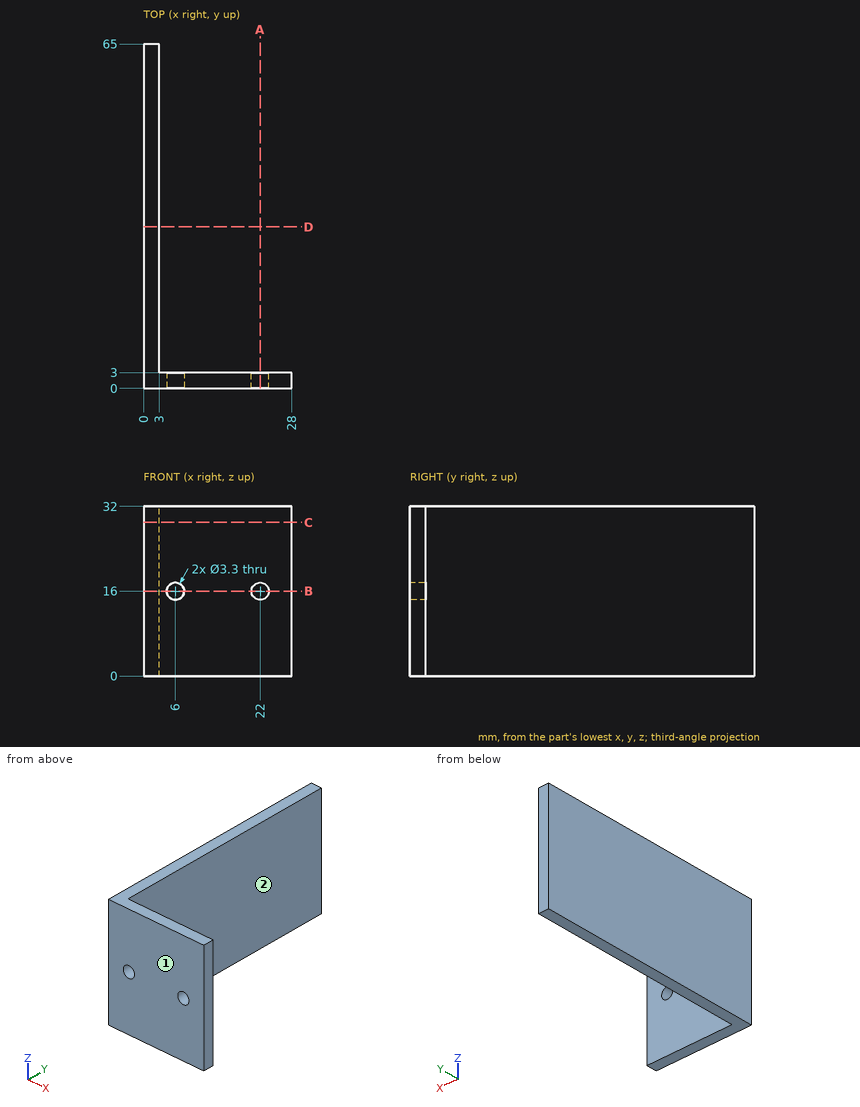
Part print with two shaded views. Sizes in mm from the minimum x, y, z corner. A direction names the side the tool comes from. Give positions to 0.01 mm unless a question says otherwise; leave off trailing zeros. Order: outer loops, then holes, each group sorted by start corner. A loop starts at its lowest first (then second) coordinate and runs counter-clockwise, first axis right, second up.
(1) Saw through at A-A, the plane x = 22. Give the cut face in (y, z), then the cut area to 3 significant figures.
(2) Flat gauge pins, fed straight in: pin 1 (7.5 mm diameter, centred on x = 11.5, z = 14.5, fed in from +Y); pin 2 (16 mm diameter, centred on y = 41, z = 23.5, fed in from +X). Where does each tip first touch, or does it go through?
(3) Saw through at C-C, the plane z = 29. Give the cut face in (x, y).
(4) Saw through at B-B, the plane z = 16. Give the cut face in (x, y).
(5) Tool access for the marked faces 1 and 2: list every direction of +Z, -Z, +X, -X, +Y, -Y with a clear straight run to the whole face (end or side of a thin tool).
(6) Saw through at D-D, the plane y = 30.5. Give the cut face in (x, z).
(7) Drill centre lines: L1, parallel to X at y = 2, z = 16; L2, parallel to Z at x = 6, y = 0.85; L3, parallel to X at y = 59.5, z = 2. Where is each one in solid material? Low to high.
Results found:
1. outline: (0, 0) - (3, 0) - (3, 14.35) - (0, 14.35) - close; (0, 17.65) - (3, 17.65) - (3, 32) - (0, 32) - close
1. area: 86.1 mm2
2. pin 1: stops at y = 3
2. pin 2: stops at x = 3
3. outline: (0, 0) - (28, 0) - (28, 3) - (3, 3) - (3, 65) - (0, 65) - close
4. outline: (0, 0) - (4.35, 0) - (4.35, 3) - (3, 3) - (3, 65) - (0, 65) - close; (7.65, 0) - (20.35, 0) - (20.35, 3) - (7.65, 3) - close; (23.65, 0) - (28, 0) - (28, 3) - (23.65, 3) - close
5. face 1: +Z, -Z, +X, -X, -Y
5. face 2: +Z, -Z, +X, +Y
6. outline: (0, 0) - (3, 0) - (3, 32) - (0, 32) - close
7. L1: x = 0 to 4.35, 7.65 to 20.35, 23.65 to 28
7. L2: z = 0 to 14.35, 17.65 to 32
7. L3: x = 0 to 3
